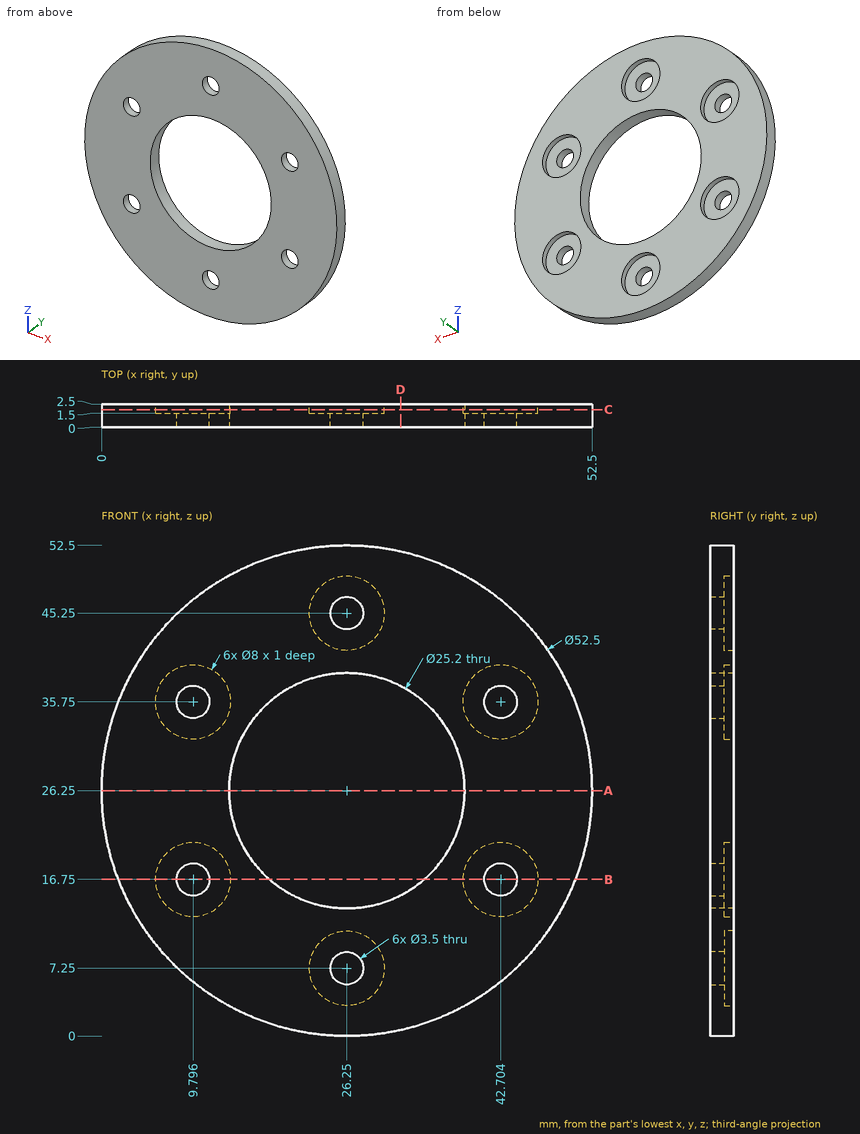
Design review of the part shown in the three views and the two pictorial views. Dimensions are in mm from the part's minimum x, y and z. Coordinates: 2 decimals unless noted, no trailing zeros. Loops run counter-clockwise (first coordinate to the right, second up) from the corner with the lowest first, then second, coordinate; pieces in that order, holes last. Notation, with made-up numbers: M -29.5,44 L -25.5,44 A9 cw -25.5,52 Z; hole C -34,64.25 d6. An arc over 180 degrees is marked long. Put each result on its own line as item: value. Start each with the question number.
Q1. Add section B-B (z = 16.75). Write out the cut boundary in (x, y) (1 decimal).
Q2. Clearance check with flat-ended pins moving along their axes: pin 1 (9 mm diameter, centred on x = 41, z = 16.5, fed in from +Y); pin 2 (6.5 mm diameter, centred on x = 26.25, z = 7.25, fed in from +Y); pin 3 (1.5 mm diameter, centred on x = 14.5, y = 2, fed in from -Z) (1 decimal); pin 4 (1.5 mm diameter, centred on y = 1.5, z = 23.5, fed in from +X). State where each tip first meets the part, or that it passes through.
Q3. Add section D-D (x = 32). Write out the cut boundary in (y, z).
Q4. Wall thickness on line 1 (X direction, y = 2.3, z = 16.75) (1 decimal); line 2 (Z direction, x = 42, y = 1.15); line 3 (Z direction, x = 42.5, y = 1.4) (1 decimal): over which ranges is each line inside the solid? List them lowest first.
Q5. Add section C-C (y = 1.9). Count the separate pieces of the cut face and the enclosed holes in it, and give its area (3 significant figures).
Q6. Add section A-A (z = 26.25). Write out the cut boundary in (x, y).
Answers:
1. outline: M 1.8,0 L 8,0 L 8,1.5 L 5.8,1.5 L 5.8,2.5 L 1.8,2.5 Z; M 11.5,0 L 18,0 L 18,2.5 L 13.8,2.5 L 13.8,1.5 L 11.5,1.5 Z; M 34.5,0 L 41,0 L 41,1.5 L 38.7,1.5 L 38.7,2.5 L 34.5,2.5 Z; M 44.5,0 L 50.7,0 L 50.7,2.5 L 46.7,2.5 L 46.7,1.5 L 44.5,1.5 Z
2. pin 1: stops at y = 2.5
2. pin 2: stops at y = 1.5
2. pin 3: stops at z = 2.4
2. pin 4: stops at x = 52.42
3. outline: M 0,0.64 L 2.5,0.64 L 2.5,15.04 L 0,15.04 Z; M 0,37.46 L 2.5,37.46 L 2.5,51.86 L 0,51.86 Z
4. line 1: x = 1.8 to 5.8, 13.8 to 18, 34.5 to 38.7, 46.7 to 50.7
4. line 2: z = 5.25 to 15.15, 18.35 to 34.15, 37.35 to 47.25
4. line 3: z = 5.6 to 15, 18.5 to 34, 37.5 to 46.9
5. separate pieces: 1
5. enclosed holes: 7
5. area: 1,360 mm^2
6. outline: M 0,0 L 13.65,0 L 13.65,2.5 L 0,2.5 Z; M 38.85,0 L 52.5,0 L 52.5,2.5 L 38.85,2.5 Z
